Geometry: see drawing. Coordinates: mm, zero at the bounding-box minimum. Coordinates: 2 decimals unless noted, no trailing zeros. Write each loop counter-clockwise with the first axis right and the second up, starting at its lowest first coordinate (ties: lowest second). Pieces come first, ordered by that corner, then holes. Notation, with made-up numbers: (-23, 39.25) - (-6, 39.25) arc R36 cw to (-6, 73.25) - close; hole circle Ø3 at (53.5, 68). An arc over 180 degrees is marked (long way). Use CSV: the item, a comma, the result in double quotes.
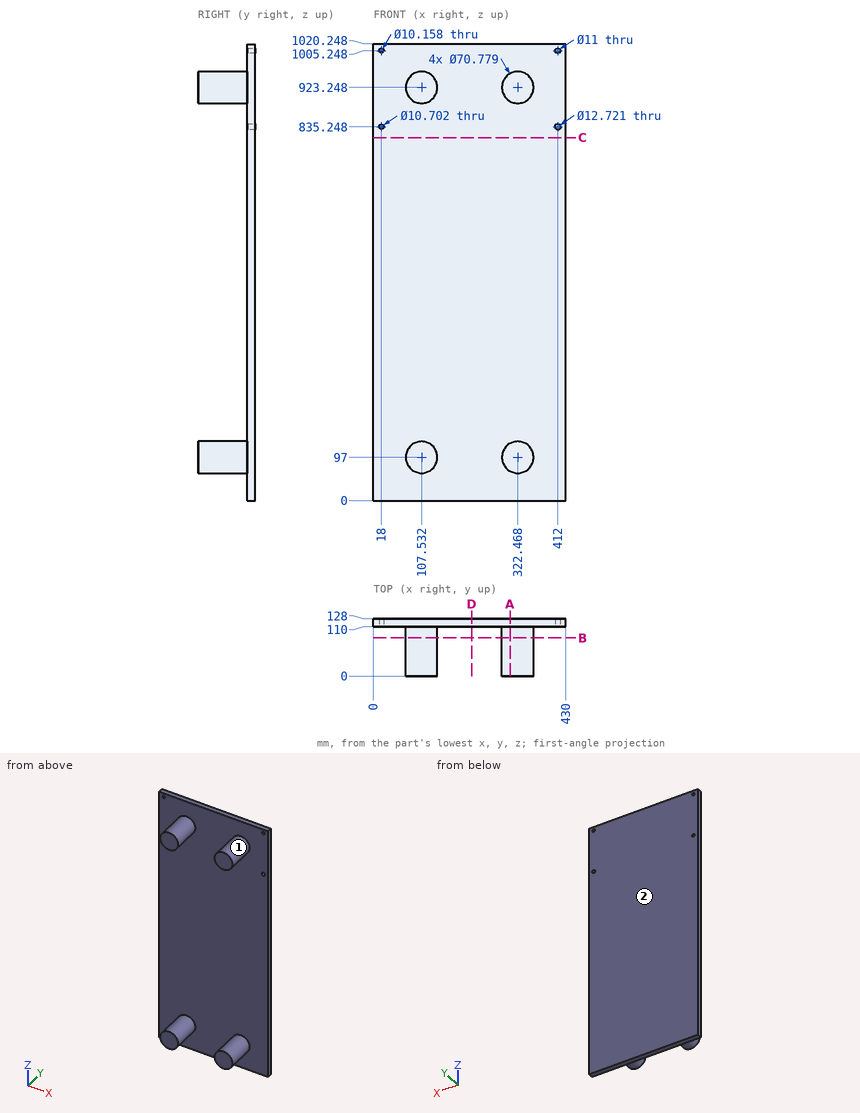
(1) Cut plane D-D on x = 219.5. Return loops of the section in (y, z).
Check values:
outline,"(110, 0) - (128, 0) - (128, 1020.25) - (110, 1020.25) - close"
(2) Cut plane C-C on z = 811. Return loops of the section in (x, y).
Check values:
outline,"(0, 110) - (430, 110) - (430, 128) - (0, 128) - close"
(3) Ray query, probe 1 along Z at (x, y) = (323, 39) (1 decimal); probe 2 along X at (y, z) = (29.5, 95.5) (1 decimal); probe 3 along Y at (x, z) = (60, 657.5). Return the intervals inside material, ascending. Write a range as from..to.
Check values:
probe 1,"61.6..132.4, 887.9..958.6"
probe 2,"72.2..142.9, 287.1..357.8"
probe 3,"110..128"
(4) Cut plane B-B on y = 85. Return loops of the section in (x, z), and give its area (3 significant figures).
Check values:
outline,"circle Ø70.78 at (107.53, 97); circle Ø70.78 at (107.53, 923.25); circle Ø70.78 at (322.47, 97); circle Ø70.78 at (322.47, 923.25)"
area,"15,700 mm^2"
(5) Draft query along Z for the marked faces 1 and 2. Return one class per face: pulls with the +Z half, pulls with the -Z half, needs draft (parallel to the pull), parting line crosses it, or undercut.
Check values:
face 1,"undercut"
face 2,"needs draft"
(6) Cut plane A-A on x = 305.5. Return loops of the section in (y, z) (1 decimal).
Check values:
outline,"(0, 65.9) - (110, 65.9) - (110, 0) - (128, 0) - (128, 1020.2) - (110, 1020.2) - (110, 954.3) - (0, 954.3) - (0, 892.2) - (110, 892.2) - (110, 128.1) - (0, 128.1) - close"
(7) Pin query (flat end, axial travel): pin 1 Ø11.5 at (x, z) = (412, 835.25) entering from +Y; pin 2 Ø1.5 at (x, z) = (54, 836.5) entering from -Y. Return the tip coordinate at first contact, or that it passes through.
Check values:
pin 1,"through"
pin 2,"y = 110"
